Geometry: final body of the model. Coordinates: model frame, mm. A direction names the side the tool comes from. Give positions to 0.01 mm unless a question says otherwise; leave off trailing zeros. Loops run counter-clockwise (first coordinate to the right, second up) from the corner with the lowest first, then second, coordinate; pieces in that order, holes last. Notation, with made-up numbers: (67.25, -36.75) - (89.25, -36.75) arc R21 ccw to (89.25, -25.75) - close; hole circle Ø3 at (35, 31.5). An arc over 180 degrees is marked (long way). Use one line per item in the form item = value.
```python
from build123d import *

# Parameters (mm, degrees)
BASE_PLATE_DEPTH   = 12
RAISED_PAD_DEPTH   = 7
HUB_BOSS_PROFILE_R = 12.512998998
HUB_BOSS_DEPTH     = 15
BORE_12_PROFILE_R  = 6
BORE_12_DEPTH      = 68


with BuildPart() as part:
    # Base Plate Profile → Base Plate (new body)
    with BuildSketch(Plane(origin=(0, 0, 0), x_dir=(1, 0, 0), z_dir=(0, 1, 0))):
        with BuildLine():
            Line((-22.062998998, 0), (-22.062998998, 35))
            Line((-22.062998998, 35), (62.937001002, 35))
            ThreePointArc((62.937001002, 35), (56.656926651, 13.374824859), (36.182547719, 4))
            Line((36.182547719, 4), (36.121903227, 4))
            ThreePointArc((36.121903227, 4), (26.759967036, 0.975135867), (20.93785397, -6.955731155))
            ThreePointArc((20.93785397, -6.955731155), (-3.52307207, -21.779896418), (-22.062998998, 0))
        make_face()
    extrude(amount=BASE_PLATE_DEPTH)

    # Raised Pad Profile → Raised Pad (add)
    with BuildSketch(Plane(origin=(0, 12, 0), x_dir=(1, 0, 0), z_dir=(0, 1, 0))):
        with BuildLine():
            Line((-12.512998998, 35), (-12.512998998, 0))
            ThreePointArc((-12.512998998, 0), (0.432197973, -12.505532729), (12.483142832, 0.863880178))
            ThreePointArc((12.483142832, 0.863880178), (16.674295928, 6.54084856), (22.899922014, 9.862792887))
            ThreePointArc((22.899922014, 9.862792887), (25.728454671, 12.778886311), (26.759967036, 16.708285768))
            Line((26.759967036, 16.708285768), (26.759967036, 35))
            Line((26.759967036, 35), (-12.512998998, 35))
        make_face()
    extrude(amount=RAISED_PAD_DEPTH)

    # Hub Boss Profile → Hub Boss (add)
    with BuildSketch(Plane(origin=(0, 19, 0), x_dir=(1, 0, 0), z_dir=(0, 1, 0))):
        with Locations(Location((0, 0, 0), (0, 0, 3.958770586))):
            Circle(HUB_BOSS_PROFILE_R)
    extrude(amount=HUB_BOSS_DEPTH)

    # Bore Ø12 Profile → Bore Ø12 (cut)
    with BuildSketch(Plane(origin=(0, 34, 0), x_dir=(1, 0, 0), z_dir=(0, 1, 0))):
        with Locations(Location((0, 0, 0), (0, 0, 270))):
            Circle(BORE_12_PROFILE_R)
    extrude(amount=-BORE_12_DEPTH, mode=Mode.SUBTRACT)


solid = part.part
```
(1) Pin query (flat end, axial travel): P1, Ø4, axis at x = -1.5, z = -27, coming from the +Y side; P2, Ø8, axis at x = 2, y = 25.5, coming from the -Z side; P3, Ø3.5, axis at y = 15, z = -27, coming from the +X side. Return the tip coordinate at first contact, or that it passes through.
Solution:
P1 = 19
P2 = -12.51
P3 = 26.76
(2) Cut plane A-A (y = 8). Return the cut outline in (x, z).
Solution:
outline = (-22.06, -35) - (62.94, -35) arc R27.05 ccw to (36.18, -4) - (36.12, -4) arc R16 cw to (20.94, 6.96) arc R22.06 ccw to (-22.06, 0) - close; hole circle Ø12 at (0, 0)
(3) Cut plane B-B (x = 0). Return the cut outline in (y, z).
Solution:
outline = (0, -35) - (19, -35) - (19, -12.51) - (34, -12.51) - (34, -6) - (0, -6) - close; (0, 6) - (34, 6) - (34, 12.51) - (12, 12.51) - (12, 22.06) - (0, 22.06) - close
(4) Pull-direction query (Z, two-part tool) for faces 1 (the face through (20, 7, -35)), 2 (the face through (26.874, 5.916, -1.057)), 3 (the face through (1.802, 17.238, 5.723)), 4 (the face through (-12.513, 15, -18)); classes: released by +Z, released by -Z, zero draft, split by the parting line, or undercut.
Solution:
face_1 = released by -Z
face_2 = released by +Z
face_3 = undercut
face_4 = zero draft
(5) Cut plane D-D (z = 9). Return the cut outline in (x, y).
Solution:
outline = (-20.14, 0) - (20.14, 0) - (20.14, 12) - (8.69, 12) - (8.69, 34) - (-8.69, 34) - (-8.69, 12) - (-20.14, 12) - close
(6) Material intervals for L1, parallel to X at y = 14, z = 0; L2, parallel to Y at x = -14, z = 0; L3, parallel to X at y = 16, z = -26, sorted ascending. Write a range as from..to.
Solution:
L1 = -12.51..-6, 6..12.51
L2 = 0..12
L3 = -12.51..26.76
(7) Access query for faces 5 (the face through (26.76, 15, -26)), 6 (the face through (21, 12, -7)), 7 (the face through (5.2, 34, -3.3)), 8 (the face through (16.599, 15.451, -6.475)). Directions: +Z, -Z, +X, -X, +Y, -Y. A direction counts if a zero-diameter tool reaches every point of the face in a straight line with its end or side. Return the directions, or none.
Solution:
face_5 = +Z, -Z, +X, +Y
face_6 = +Z, +Y
face_7 = +Z, -Z, +X, -X, +Y
face_8 = +Z, +X, +Y
(8) Cut plane C-C (z = 3). Return the cut outline in (x, y), plus the area to 3 significant figures.
Solution:
outline = (-21.86, 0) - (-5.2, 0) - (-5.2, 34) - (-12.15, 34) - (-12.15, 12) - (-21.86, 12) - close; (5.2, 0) - (22.89, 0) - (22.89, 12) - (12.15, 12) - (12.15, 34) - (5.2, 34) - close
area = 718 mm2
